For this review, take the finished solid that the model builds, in its own axes (mm). Coordinates: 2 decimals unless noted, no trailing zeros. Order: outer loops, then holes, each group sorted by start corner. A loop starts at its lowest first (then second) coordinate and runs counter-clockwise, first axis right, second up. Notation, with made-up numbers: (15.25, 74) -> (46.25, 74) arc R20 cw to (46.25, 80) -> close; hole circle Ø4 at (32, 4.25). An arc over 180 degrees is marked (long way). Write item = value, one per line. Start each with the question number.
1) Consider section B-B on z = -15. State how many separate pieces and enclosed holes the cut face has, and give its area (3 significant figures).
2) Consider section A-A on x = -25. Give the boundary of the cut face in (y, z), and give its area (3 significant figures).
3) Insertion check: pin 1 Ø6 at (x, z) = (47.5, 0.5) entering from -Y; pin 2 Ø5 at (x, z) = (-26, 15) entering from -Y. Each pin has a flat end and moves straight along its axis. Give the tip position at first contact, or say it passes through.
4) Consider section D-D on x = -45.5. Give the boundary of the cut face in (y, z), and give its area (3 significant figures).
5) Wall thickness on probe 1 along Z at (x, y) = (0, 6); probe 2 along Z at (x, y) = (-24.5, 4): over which ranges is each line inside the solid? List them lowest first. Write a range as [from, to].
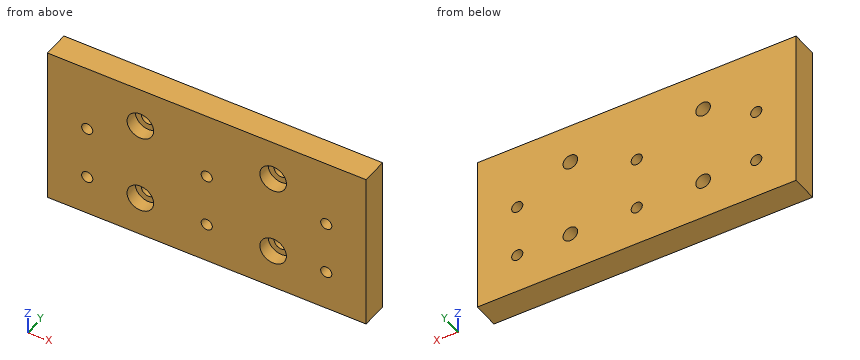
from build123d import *

# Parameters (mm, degrees)
SKETCH_1_W                                         = 120
SKETCH_1_H                                         = 60
BOSS_EXTRUDE_1_DEPTH                               = 10
M5_SOCKET_HEAD_CAP_SCREW_COUNTERBORE_1_D           = 5.5
M5_SOCKET_HEAD_CAP_SCREW_COUNTERBORE_1_CBORE_D     = 10
M5_SOCKET_HEAD_CAP_SCREW_COUNTERBORE_1_CBORE_DEPTH = 5
LINEAR_PATTERN_1_COUNT                             = 2
LINEAR_PATTERN_1_PITCH                             = 50
LINEAR_PATTERN_1_COUNT_DIR2                        = 2
LINEAR_PATTERN_1_PITCH_DIR2                        = 30
M5_TAPPED_HOLE_1_D                                 = 4.2
LINEAR_PATTERN_2_COUNT                             = 2
LINEAR_PATTERN_2_PITCH                             = 20
LINEAR_PATTERN_2_COUNT_DIR2                        = 3
LINEAR_PATTERN_2_PITCH_DIR2                        = 45


with BuildPart() as part:
    # Sketch 1 → Boss-Extrude 1 (new body)
    with BuildSketch(Plane(origin=(0, 0, 0), x_dir=(1, 0, 0), z_dir=(0, 1, 0))):
        Rectangle(SKETCH_1_W, SKETCH_1_H)
    extrude(amount=BOSS_EXTRUDE_1_DEPTH)

    # M5 Socket Head Cap Screw Counterbore 1 (through all)
    with Locations(Plane.XZ):
        with Locations((-25, 15)):
            m5_socket_head_cap_screw_counterbore_1 = CounterBoreHole(M5_SOCKET_HEAD_CAP_SCREW_COUNTERBORE_1_D / 2, M5_SOCKET_HEAD_CAP_SCREW_COUNTERBORE_1_CBORE_D / 2, M5_SOCKET_HEAD_CAP_SCREW_COUNTERBORE_1_CBORE_DEPTH)

    # Linear Pattern 1: M5 Socket Head Cap Screw Counterbore 1 2 × 2
    with Locations(*[(i * LINEAR_PATTERN_1_PITCH, 0, -j * LINEAR_PATTERN_1_PITCH_DIR2) for i in range(LINEAR_PATTERN_1_COUNT) for j in range(LINEAR_PATTERN_1_COUNT_DIR2) if (i, j) != (0, 0)]):
        add(m5_socket_head_cap_screw_counterbore_1, mode=Mode.SUBTRACT)

    # M5 Tapped Hole 1 (through all)
    with Locations(Plane.XZ):
        with Locations((-45, 5)):
            m5_tapped_hole_1 = Hole(M5_TAPPED_HOLE_1_D / 2)

    # Linear Pattern 2: M5 Tapped Hole 1 2 × 3
    with Locations(*[(j * LINEAR_PATTERN_2_PITCH_DIR2, 0, -i * LINEAR_PATTERN_2_PITCH) for i in range(LINEAR_PATTERN_2_COUNT) for j in range(LINEAR_PATTERN_2_COUNT_DIR2) if (i, j) != (0, 0)]):
        add(m5_tapped_hole_1, mode=Mode.SUBTRACT)


solid = part.part
Answer sheet:
q1.separate_pieces = 6
q1.enclosed_holes = 0
q1.area = 919 mm2
q2.outline = (0, -30) -> (10, -30) -> (10, -17.75) -> (5, -17.75) -> (5, -20) -> (0, -20) -> close; (0, -10) -> (5, -10) -> (5, -12.25) -> (10, -12.25) -> (10, 12.25) -> (5, 12.25) -> (5, 10) -> (0, 10) -> close; (0, 20) -> (5, 20) -> (5, 17.75) -> (10, 17.75) -> (10, 30) -> (0, 30) -> close
q2.area = 445 mm2
q3.pin_1 = 0
q3.pin_2 = 5
q4.outline = (0, -30) -> (10, -30) -> (10, -17.04) -> (0, -17.04) -> close; (0, -12.96) -> (10, -12.96) -> (10, 2.96) -> (0, 2.96) -> close; (0, 7.04) -> (10, 7.04) -> (10, 30) -> (0, 30) -> close
q4.area = 518 mm2
q5.probe_1 = [-30, -17.1], [-12.9, 2.9], [7.1, 30]
q5.probe_2 = [-30, -19.97], [-10.03, 10.03], [19.97, 30]
